Could you check a few things on this drawing? It's one solid part, dimensions in mm from its lowest x, y, z. A direction names the side the tool comes from. Give positions to 0.01 mm unless a question says otherwise; leave off trailing zeros. Order: outer loops, then holes, each group sorted by start corner. A loop starts at its lowest first (then second) coordinate and runs counter-clockwise, first axis right, second up.
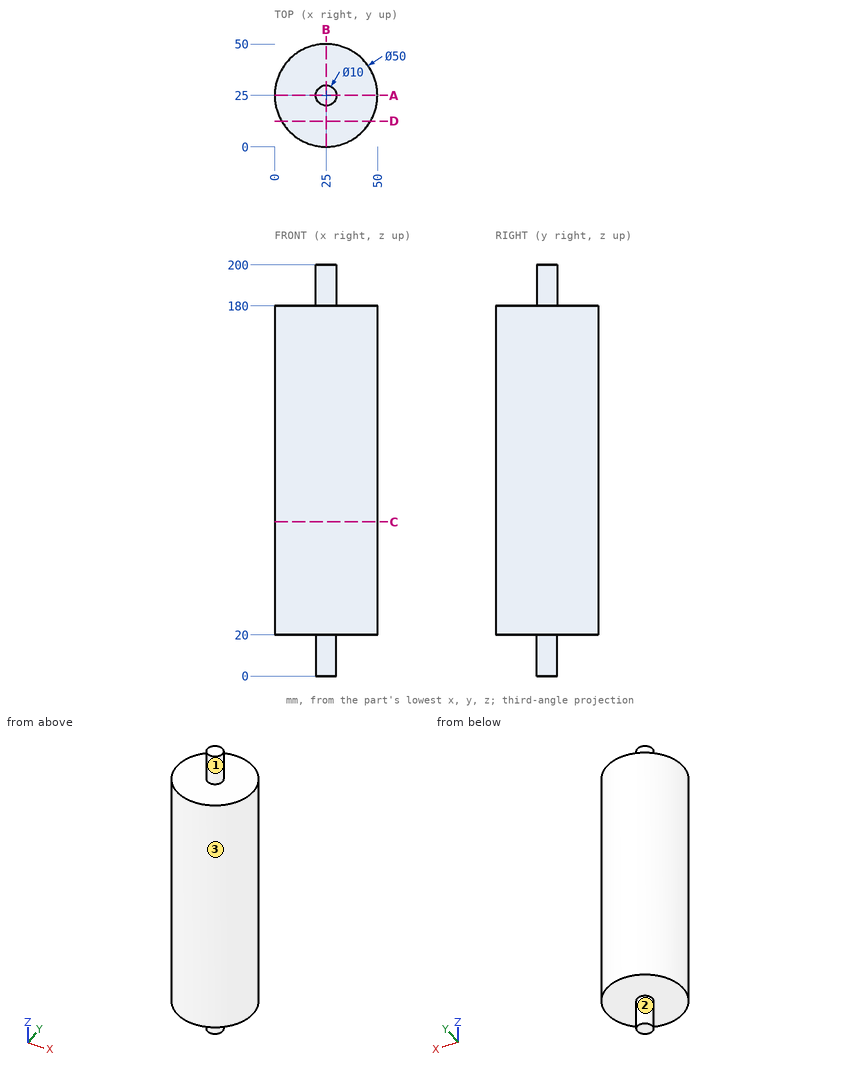
Q1. I need wall thicknesses on L1, parallel to Y at x = 25, z = 21; L2, parallel to Z at x = 42, y = 29; L3, parallel to X at y = 25.5, z = 42.5 (3 decimals). Which ranges of each line are inside material? Lowest first, please.
Filled sheet:
L1: y = 0 to 50
L2: z = 20 to 180
L3: x = 0.005 to 49.995
Q2. I'm going to push flat-ended pins straight in: P1, Ø6, axis at x = 10, z = 20.5, coming from the +Y side; P2, Ø12, axis at x = 18.5, z = 166, coming from the -Y side (3 decimals); P3, Ø6, axis at x = 22.5, z = 153.5, coming from the +Y side. Where does each tip first touch, or does it pass through?
Filled sheet:
P1: stops at y = 46.93
P2: stops at y = 0.005
P3: stops at y = 50
Q3. For the marked faces 1, 2 and 3, which set-ups out of +Z, -Z, +X, -X, +Y, -Y let a thin tool reach every point of the face, with its end or its side?
Filled sheet:
face 1: +Z
face 2: -Z
face 3: +Z, -Z
Q4. If we section it at D-D on y = 12.5: List the corners of the cut face in (x, z) for me, plus the area to 3 significant figures.
Filled sheet:
outline: (3.35, 20) - (46.65, 20) - (46.65, 180) - (3.35, 180) - close
area: 6,930 mm2
Q5. If we section it at A-A on y = 25: List the corners of the cut face in (x, z) for me.
Filled sheet:
outline: (0, 20) - (20, 20) - (20, 0) - (30, 0) - (30, 20) - (50, 20) - (50, 180) - (30, 180) - (30, 200) - (20, 200) - (20, 180) - (0, 180) - close
Q6. If we section it at C-C on z = 75: List the corners of the cut face in (x, y) for me.
Filled sheet:
outline: circle Ø50 at (25, 25)
